Answer from the drawing. Dimensions are ordinates in mm from the lowest x, y and z of the part. A direction names the side the tool comes from. Give positions to 0.01 mm unless a question says otherwise; leave off trailing zeros. Order: outer loops, then holes, each group sorted by start corner. A loop starts at its lowest first (then second) coordinate and runs counter-clockwise, first axis right, second up. Notation, with made-up numbers: (20, 71.25) -> (52, 71.25) arc R7 cw to (52, 77.25) -> close; hole circle Ø4 at (25, -9.75). An arc over 180 degrees is marked (long way). Answer as CSV lines item,"result". Start each with the question number.
1) For the marked faces 4, 5, 6, 7 and 8, determine the directions among +Z, -Z, +X, -X, +Y, -Y from which every point of the face is accessible in a straight line to the end or side of a thin tool.
2) Flat-ended cylindrical pins translate along their axes: pin 1 Ø6 at (x, y) = (31.5, 37) entering from +Z; pin 2 Ø9 at (x, z) = (5.5, 18.5) entering from -Y; pin 3 Ø2 at (x, z) = (23.5, 3) entering from +Y; pin 4 Ø5 at (x, y) = (28, 37.5) entering from +Z. Find the tip coordinate at first contact, or state that the pin passes through.
3) Find section D-D (y = 16). Determine the outline of the cut face in (x, z) (1 decimal), and give its area (3 significant figures).
4) Straight lines are drawn through the part: L1, parallel to Y at x = 13, z = 27.5; L2, parallel to X at y = 40, z = 24; L3, parallel to Y at x = 28.5, z = 6. For each, find the intervals that lie inside material, in ascending order. Write a range as from..to.
5) Find section C-C (y = 40). Determine the outline of the cut face in (x, z), and give its area (3 significant figures).
6) The mould has two halves that part along X. Classify the marked faces 1, 2 and 3: +X half, -X half, draft (parallel to the pull), parting line (faces both ways), or undercut.
7) Find section B-B (x = 27). Determine the outline of the cut face in (y, z), and give its area (3 significant figures).
8) Find section A-A (z = 16). Determine the outline of the cut face in (x, y), and give its area (3 significant figures).
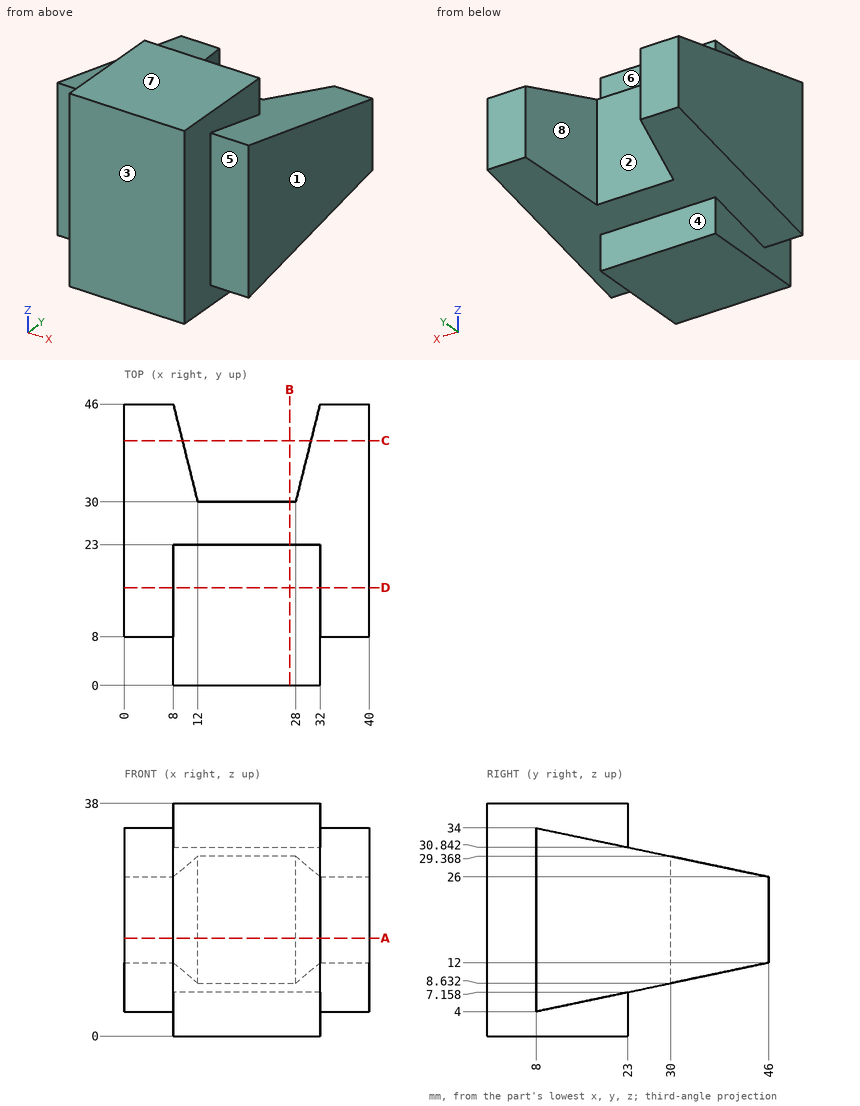
Findings below:
1,face 4,"-Z, +X, -X, +Y"
1,face 5,"+Z, -Z, +X, -Y"
1,face 6,"+Z, +X, -X, +Y"
1,face 7,"+Z, +X, -X, +Y, -Y"
1,face 8,"+Z, -Z, +Y"
2,pin 1,"z = 28.53"
2,pin 2,"y = 0"
2,pin 3,"y = 23"
2,pin 4,"z = 28.23"
3,outline,"(0, 5.7) -> (8, 5.7) -> (8, 0) -> (32, 0) -> (32, 5.7) -> (40, 5.7) -> (40, 32.3) -> (32, 32.3) -> (32, 38) -> (8, 38) -> (8, 32.3) -> (0, 32.3) -> close"
3,area,"1,340 mm²"
4,L1,"0..30"
4,L2,"0..9.5, 30.5..40"
4,L3,"0..23"
5,outline,"(0, 10.74) -> (9.5, 10.74) -> (9.5, 27.26) -> (0, 27.26) -> close; (30.5, 10.74) -> (40, 10.74) -> (40, 27.26) -> (30.5, 27.26) -> close"
5,area,"314 mm²"
6,face 1,"+X half"
6,face 2,"undercut"
6,face 3,"draft"
7,outline,"(0, 0) -> (23, 0) -> (23, 7.16) -> (30, 8.63) -> (30, 29.37) -> (23, 30.84) -> (23, 38) -> (0, 38) -> close"
7,area,"1,030 mm²"
8,outline,"(0, 8) -> (8, 8) -> (8, 0) -> (32, 0) -> (32, 8) -> (40, 8) -> (40, 46) -> (32, 46) -> (28, 30) -> (12, 30) -> (8, 46) -> (0, 46) -> close"
8,area,"1,390 mm²"
